```python
from build123d import *

# Parameters (mm, degrees)
SKETCH_1_W                = 101
SKETCH_1_H                = 130
EXTRUDE_1_DEPTH           = 11
CUT_EXTRUDE_1_DEPTH       = 8
CUT_EXTRUDE_2_DEPTH       = 8
CUT_EXTRUDE_3_REACH       = 1271.625
SKETCH_4_W                = 4
SKETCH_4_H                = 32
CUT_EXTRUDE_4_REACH       = 1273.161
SKETCH_5_W                = 4
SKETCH_5_H                = 32
SKETCH_6_R                = 36
EXTRUDE_2_DEPTH           = 5
SKETCH_7_R                = 18
EXTRUDE_3_DEPTH           = 6
SKETCH_8_R                = 32
CUT_EXTRUDE_5_DEPTH       = 5
SKETCH_9_R                = 13
CUT_EXTRUDE_6_DEPTH       = 6.5
SKETCH_10_R               = 10
CUT_EXTRUDE_7_DEPTH       = 0.5
SKETCH_11_R               = 5.25
CUT_EXTRUDE_8_DEPTH       = 97.916510461
HOLE_WIZARD_7_0_7_1_D     = 7
HOLE_WIZARD_7_0_7_1_DEPTH = 22
FILLET_1_R                = 5
CHAMFER_1_SIZE            = 1
FILLET_2_R                = 2
FILLET_3_R                = 3
FILLET_4_R                = 4
FILLET_5_R                = 10


with BuildPart() as part:
    # 草图1 → 凸台-拉伸1 (new body)
    with BuildSketch(Plane(origin=(1263, 0, 0), x_dir=(0, 0, -1), z_dir=(1, 0, 0))):
        with Locations((-11, -6.6)):
            Rectangle(SKETCH_1_W, SKETCH_1_H)
    extrude(amount=-EXTRUDE_1_DEPTH)

    # 草图2 → 切除-拉伸1 (cut)
    with BuildSketch(Plane(origin=(1263, 0, 0), x_dir=(0, 0, -1), z_dir=(1, 0, 0))):
        with BuildLine():
            Line((14.5, 42.4), (-44.5, 42.4))
            Line((-44.5, 42.4), (-44.5, 25.256406461))
            ThreePointArc((-44.5, 25.256406461), (-48.17544468, 17.510439768), (-56.5, 15.458447489))
            Line((-56.5, 15.458447489), (-56.5, -48.6))
            ThreePointArc((-56.5, -48.6), (-51.227922061, -61.327922061), (-38.5, -66.6))
            Line((-38.5, -66.6), (16.5, -66.6))
            ThreePointArc((16.5, -66.6), (29.227922061, -61.327922061), (34.5, -48.6))
            Line((34.5, -48.6), (34.5, 15.4))
            Line((34.5, 15.4), (14.5, 15.4))
            Line((14.5, 15.4), (14.5, 42.4))
        make_face()
    extrude(amount=-CUT_EXTRUDE_1_DEPTH, mode=Mode.SUBTRACT)

    # 草图3 → 切除-拉伸2 (cut)
    with BuildSketch(Plane(origin=(1263, 0, 0), x_dir=(0, 0, -1), z_dir=(1, 0, 0))):
        with BuildLine():
            Line((20, 55.4), (-42, 55.4))
            ThreePointArc((-42, 55.4), (-47, 50.4), (-42, 45.4))
            Line((-42, 45.4), (20, 45.4))
            ThreePointArc((20, 45.4), (25, 50.4), (20, 55.4))
        make_face()
    extrude(amount=-CUT_EXTRUDE_2_DEPTH, mode=Mode.SUBTRACT)

    # 草图4 → 切除-拉伸3 (cut, up to next)
    with BuildSketch(Plane.XZ.offset(-42.4), mode=Mode.PRIVATE) as cut_extrude_3_sk1:
        with Locations((1261, 11)):
            Rectangle(SKETCH_4_W, SKETCH_4_H)
    cut_extrude_3_tool1 = extrude(cut_extrude_3_sk1.sketch, amount=-CUT_EXTRUDE_3_REACH, mode=Mode.PRIVATE) & part.part
    add(cut_extrude_3_tool1.solids().sort_by_distance((1261, 42.4, 11))[0], mode=Mode.SUBTRACT)

    # 草图5 → 切除-拉伸4 (cut, up to next)
    with BuildSketch(Plane(origin=(0, 58.4, 0), x_dir=(-1, 0, 0), z_dir=(0, 1, 0)), mode=Mode.PRIVATE) as cut_extrude_4_sk1:
        with Locations((-1261, 11)):
            Rectangle(SKETCH_5_W, SKETCH_5_H)
    cut_extrude_4_tool1 = extrude(cut_extrude_4_sk1.sketch, amount=-CUT_EXTRUDE_4_REACH, mode=Mode.PRIVATE) & part.part
    add(cut_extrude_4_tool1.solids().sort_by_distance((1261, 58.4, 11))[0], mode=Mode.SUBTRACT)

    # 草图6 → 凸台-拉伸2 (add)
    with BuildSketch(Plane.ZY.offset(-1252)):
        with Locations((11, -25.6)):
            Circle(SKETCH_6_R)
    extrude(amount=EXTRUDE_2_DEPTH)

    # 草图7 → 凸台-拉伸3 (add)
    with BuildSketch(Plane.ZY.offset(-1247)):
        with Locations((11, -25.6)):
            Circle(SKETCH_7_R)
    extrude(amount=EXTRUDE_3_DEPTH)

    # 草图8 → 切除-拉伸5 (cut)
    with BuildSketch(Plane(origin=(1255, 0, 0), x_dir=(0, 0, -1), z_dir=(1, 0, 0))):
        with Locations(Location((-11, -25.6, 0), (0, 0, 180))):
            Circle(SKETCH_8_R)
    extrude(amount=-CUT_EXTRUDE_5_DEPTH, mode=Mode.SUBTRACT)

    # 草图9 → 切除-拉伸6 (cut)
    with BuildSketch(Plane(origin=(1250, 0, 0), x_dir=(0, 0, -1), z_dir=(1, 0, 0))):
        with Locations(Location((-11, -25.6, 0), (0, 0, 180))):
            Circle(SKETCH_9_R)
    extrude(amount=-CUT_EXTRUDE_6_DEPTH, mode=Mode.SUBTRACT)

    # 草图10 → 切除-拉伸7 (cut)
    with BuildSketch(Plane(origin=(1243.5, 0, 0), x_dir=(0, 0, -1), z_dir=(1, 0, 0))):
        with Locations(Location((-11, -25.6, 0), (0, 0, 180))):
            Circle(SKETCH_10_R)
    extrude(amount=-CUT_EXTRUDE_7_DEPTH, mode=Mode.SUBTRACT)

    # 草图11 → 切除-拉伸8 (cut, through all)
    with BuildSketch(Plane.ZY.offset(-1241)):
        with Locations((11, -25.6)):
            Circle(SKETCH_11_R)
    extrude(amount=-CUT_EXTRUDE_8_DEPTH, mode=Mode.SUBTRACT)

    # Ø7.0 (7) 直径孔1
    with Locations(Plane(origin=(1263, 0, 0), x_dir=(0, 0, -1), z_dir=(1, 0, 0))):
        with Locations((-55.5, -65.6), (33.5, -65.6), (25.5, 21.4), (25.5, 41.4), (-53.5, 41.4), (-53.5, 21.4)):
            Hole(HOLE_WIZARD_7_0_7_1_D / 2, depth=HOLE_WIZARD_7_0_7_1_DEPTH)

    # 圆角1
    fillet_1_edges = [part.edges().sort_by_distance(p)[0] for p in [
        (1257.5, -71.6, -39.5),
        (1257.5, -71.6, 61.5),
        (1257.5, 58.4, 61.5),
        (1257.5, 58.4, -39.5),
    ]]
    fillet(fillet_1_edges, radius=FILLET_1_R)

    # 倒角1
    chamfer_1_edges = [part.edges().sort_by_distance(p)[0] for p in [
        (1252, 58.4, 11),
        (1252, -6.6, 61.5),
        (1252, -6.6, -39.5),
        (1252, -71.6, 11),
        (1252, -70.135533906, 60.035533906),
        (1252, -70.135533906, -38.035533906),
        (1252, 56.935533906, -38.035533906),
        (1252, 56.935533906, 60.035533906),
        (1255, -25.6, -21),
        (1250, -25.6, -2),
    ]]
    chamfer(chamfer_1_edges, length=CHAMFER_1_SIZE)

    # 圆角2
    fillet_2_edges = [part.edges().sort_by_distance(p)[0] for p in [
        (1252, -25.6, -25),
        (1247, -25.6, -25),
        (1247, -25.6, -7),
    ]]
    fillet(fillet_2_edges, radius=FILLET_2_R)

    # 圆角3
    fillet_3_edges = [part.edges().sort_by_distance(p)[0] for p in [
        (1241, -25.6, -7),
    ]]
    fillet(fillet_3_edges, radius=FILLET_3_R)

    # 圆角4
    fillet_4_edges = [part.edges().sort_by_distance(p)[0] for p in [
        (1259, 42.4, -14.5),
        (1259, 15.4, -34.5),
        (1259, 15.458447489, 56.5),
        (1259, 42.4, 44.5),
    ]]
    fillet(fillet_4_edges, radius=FILLET_4_R)

    # 圆角5
    fillet_5_edges = [part.edges().sort_by_distance(p)[0] for p in [
        (1259, 15.4, -14.5),
    ]]
    fillet(fillet_5_edges, radius=FILLET_5_R)


solid = part.part
```
Check sheet for the modelled part. Datum: model origin and axes. Units: mm. A direction names the side the tool comes from. Round coordinates to 2 decimals unless told otherwise and drop trailing zeros. Loops run counter-clockwise (first coordinate to the right, second up) from the corner with the lowest first, then second, coordinate; pieces in that order, holes last. Notation, with made-up numbers: M 72,14 L 84,14 A31 ccw 84,50 Z; hole C -34,-26 d4. An arc over 180 degrees is marked long. Answer as a JSON object with one key per item and string values.
1. Section check B-B (y = 50.4). Record the boundary of the cut face in (x, z), plus the area to 3 significant figures.
Reply:
{"outline": "M 1252,-38.5 L 1253,-39.5 L 1263,-39.5 L 1263,-25 L 1255,-25 L 1255,47 L 1263,47 L 1263,61.5 L 1253,61.5 L 1252,60.5 Z", "area": "534 mm²"}
2. Section check A-A (z = 54.5). Record the boundary of the cut face in (x, y), plus the area to 3 significant figures.
Reply:
{"outline": "M 1252,-70.6 L 1253,-71.6 L 1263,-71.6 L 1263,-68.95 L 1252,-68.95 Z; M 1252,-62.25 L 1263,-62.25 L 1263,-56.85 L 1255,-56.85 L 1255,14.86 L 1263,14.86 L 1263,18.05 L 1252,18.05 Z; M 1252,24.75 L 1263,24.75 L 1263,38.05 L 1252,38.05 Z; M 1252,44.75 L 1263,44.75 L 1263,58.4 L 1253,58.4 L 1252,57.4 Z", "area": "634 mm²"}
3. Access from +Z, -Z, +X, -X, +Y, -Y to the whole of each face (thin tool, end or side, straight path). Record for faces 4 (the flat face through (1261, 57, -5)), 5 (the cylindrical face through (1257.423, 20.059, -22.267)), 6 (the flat face through (1250, -12, 18)), 7 (the cylindrical face through (1257.93, -70.17, -38)), 8 (the cylindrical face through (1249.507, -47.505, -17.568)).
Reply:
{"face 4": "+X, +Y", "face 5": "+X, -X", "face 6": "+X", "face 7": "-Z, +X, -X, -Y", "face 8": "-X"}
4. Gauge pin test, flat ends, axial feed: P1, Ø2.5, axis at x = 1261, y = 57.5, coming from the +Z side; P2, Ø4, axis at x = 1251.5, z = 17, coming from the +Y side; P3, Ø6.5, axis at y = -65.6, z = -33.5, coming from the -X side; P4, Ø22, axis at y = -21.5, z = 10.5, coming from the +X side. Record the tip position at first contact, or that the pin passes through.
Reply:
{"P1": "stops at z = 60.61", "P2": "stops at y = 58.4", "P3": "passes through", "P4": "stops at x = 1250"}
5. Scan lines: line 1 (Y direction, x = 1257.5, z = -2); line 2 (Y direction, x = 1252.85, z = 11); line 3 (X direction, y = 52, z = 42.5). Record each from-to range of solid material in increasing order.
Reply:
{"line 1": "y = -71.6 to -66.6, 42.4 to 45.4, 55.4 to 58.4", "line 2": "y = -71.45 to -57.6, 6.4 to 58.25", "line 3": "x = 1252 to 1255"}
6. Mould release check, pull along X, two halves, no side actions. Record for faces 1 (the cylindrical face through (1257.4, -67.7, 52.7)), 2 (the flat face through (1243.5, -18, 18)), 3 (the flat face through (1241, -32, 11)): pulls with the +X half, pulls with the -X half, needs draft (parallel to the pull), parting line crosses it, or undercut.
Reply:
{"face 1": "needs draft", "face 2": "pulls with the +X half", "face 3": "pulls with the -X half"}
